```python
from build123d import *

# Parameters (mm, degrees)
SKETCH_1_R                = 18
SKETCH_1_R_2              = 11
EXTRUDE_1_DEPTH           = 25
SKETCH_2_R                = 29
SKETCH_2_R_2              = 11
EXTRUDE_2_DEPTH           = 15
HOLE_WIZARD_1_D           = 4.5
HOLE_WIZARD_1_CBORE_D     = 8
HOLE_WIZARD_1_CBORE_DEPTH = 4.6
SKETCH_6_W                = 24
SKETCH_6_H                = 35
CUT_EXTRUDE_1_DEPTH       = 8
EXTRUDE_START             = -5
SKETCH_7_R                = 11
SKETCH_7_R_2              = 6
EXTRUDE_3_DEPTH           = 5


with BuildPart() as part:
    # 草图1 → 凸台-拉伸1 (new body)
    with BuildSketch(Plane.XY):
        Circle(SKETCH_1_R)
        Circle(SKETCH_1_R_2, mode=Mode.SUBTRACT)
    extrude(amount=EXTRUDE_1_DEPTH)

    # 草图2 → 凸台-拉伸2 (add)
    with BuildSketch(Plane.XY.offset(25)):
        Circle(SKETCH_2_R)
        Circle(SKETCH_2_R_2, mode=Mode.SUBTRACT)
    extrude(amount=EXTRUDE_2_DEPTH)

    # 打孔尺寸根据内六角圆柱头螺钉的类型1 (through all)
    with Locations(Plane(origin=(0, 0, 25), x_dir=(-1, 0, 0), z_dir=(0, 0, -1))):
        with Locations((-23, 0), (23, 0)):
            CounterBoreHole(HOLE_WIZARD_1_D / 2, HOLE_WIZARD_1_CBORE_D / 2, HOLE_WIZARD_1_CBORE_DEPTH)

    # 草图6 → 切除-拉伸1 (cut)
    with BuildSketch(Plane.XY.offset(40)):
        Rectangle(SKETCH_6_W, SKETCH_6_H)
    extrude(amount=-CUT_EXTRUDE_1_DEPTH, mode=Mode.SUBTRACT)

    # 草图7 → 凸台-拉伸3 (add)
    with BuildSketch(Plane.XY.offset(32).offset(EXTRUDE_START)):
        Circle(SKETCH_7_R)
        Circle(SKETCH_7_R_2, mode=Mode.SUBTRACT)
    extrude(amount=EXTRUDE_3_DEPTH)


solid = part.part
```
Could you check a few things on this model? Use its own coordinates, in mm. A direction names the side the tool comes from. Give positions to 0.01 mm unless a question says otherwise; leave off trailing zeros. Order: outer loops, then holes, each group sorted by start corner. A loop starts at its lowest first (then second) coordinate and runs counter-clockwise, first axis right, second up.
Q1. Suppose I cut it at C-C, the plane z = 36. Write out the boundary of the cut face in (x, y), and give its area (3 significant figures).
Q2. If I drill on line 1 along X through (y, z) = (-1, 38.5); line 2 along Y through (x, z) = (0, 28.8); line 3 along Z through (x, y) = (-15, -17), over which ranges is the centre line in solid material (lowest first)?
Q3. Suppose I cut it at A-A, the plane x = 0. Write out the boundary of the cut face in (y, z).
Q4. For faces 5 (the flat face through (-25, -2, 29.6)), 6 (the cylindrical face through (-6, 0, 29)), 7 (the flat face through (0, 17.5, 36)), which set-ups out of +Z, -Z, +X, -X, +Y, -Y let a thin tool reach every point of the face, with its end or its side?
Q5. Suppose I cut it at B-B, the plane y = 0. Count the separate pieces of the cut face and the enclosed holes in it, and give its area (3 significant figures).
Q6. We'd pull the mould along Y, two halves only. Please class faces 1 (the flat face through (5, 4, 32)), 2 (the flat face through (12.5, 0.4, 40)), 3 (the cylindrical face through (13.38, -25.73, 32.39)), 4 (the cylindrical face through (-20.854, 0.676, 34.873)): +Y half, -Y half, draft (parallel to the pull), parting line (faces both ways), or undercut.
Q7. I'm going to push flat-ended pins straight in: P1, Ø8, axis at x = 7, z = 35.5, coming from the +Y side; P2, Ø10, axis at y = 18.5, z = 28, coming from the -X side; P3, Ø17.5, axis at x = 0, y = 0, coming from the -Z side. Where does each tip first touch, or does it pass through?
Q8. Suppose I cut it at D-D, the plane z = 17. Write out the boundary of the cut face in (x, y).
Solution:
1. outline: circle Ø58 at (0, 0); hole circle Ø4.5 at (-23, 0); hole (-12, -17.5) - (12, -17.5) - (12, 17.5) - (-12, 17.5) - close; hole circle Ø4.5 at (23, 0)
1. area: 1,770 mm2
2. line 1: x = -28.98 to -25.02, -20.98 to -12, 12 to 20.98, 25.02 to 28.98
2. line 2: y = -29 to -6, 6 to 29
2. line 3: z = 25 to 40
3. outline: (-29, 25) - (-18, 25) - (-18, 0) - (-11, 0) - (-11, 27) - (-6, 27) - (-6, 32) - (-17.5, 32) - (-17.5, 40) - (-29, 40) - close; (6, 27) - (11, 27) - (11, 0) - (18, 0) - (18, 25) - (29, 25) - (29, 40) - (17.5, 40) - (17.5, 32) - (6, 32) - close
4. face 5: -Z
4. face 6: +Z, -Z
4. face 7: +Z
5. separate pieces: 4
5. enclosed holes: 0
5. area: 757 mm2
6. face 1: undercut
6. face 2: draft
6. face 3: parting line
6. face 4: undercut
7. P1: stops at y = 28.84
7. P2: stops at x = -25.67
7. P3: stops at z = 27
8. outline: circle Ø36 at (0, 0); hole circle Ø22 at (0, 0)
